from build123d import *

# Parameters (mm, degrees)
SKETCH3_W                                            = 50
SKETCH3_H                                            = 86
SKETCH3_R                                            = 14
BOSS_EXTRUDE1_DEPTH                                  = 21
M3_TAPPED_HOLE1_D                                    = 2.5
M3_TAPPED_HOLE1_DEPTH                                = 10
M3_TAPPED_HOLE1_TIP                                  = 0.751075774
BOSS_EXTRUDE3_START                                  = -2
SKETCH4_R                                            = 14
SKETCH4_R_2                                          = 12
BOSS_EXTRUDE3_DEPTH                                  = 2
F_4_0_4_DIAMETER_HOLE2_D                             = 4
SKETCH22_W                                           = 50
SKETCH22_H                                           = 15
BOSS_EXTRUDE5_DEPTH                                  = 20
SKETCH23_R                                           = 3.25
CUT_EXTRUDE3_DEPTH                                   = 92.989129793
F_4_0_4_DIAMETER_HOLE1_D                             = 4
F_4_0_4_DIAMETER_HOLE1_DEPTH                         = 15
F_4_0_4_DIAMETER_HOLE1_TIP                           = 1.201721238
HOLE_SIZE_PER_SOCKET_HEAD_CAP_SCREW_TYPE_D           = 4.5
HOLE_SIZE_PER_SOCKET_HEAD_CAP_SCREW_TYPE_CBORE_D     = 8
HOLE_SIZE_PER_SOCKET_HEAD_CAP_SCREW_TYPE_CBORE_DEPTH = 4.6
CHAMFER1_SIZE                                        = 3
CHAMFER2_SIZE                                        = 1


with BuildPart() as part:
    # Sketch3 → Boss-Extrude1 (new body)
    with BuildSketch(Plane.XY):
        with Locations((0, 43)):
            Rectangle(SKETCH3_W, SKETCH3_H)
        with Locations(Location((0, 60, 0), (0, 0, 180))):
            Circle(SKETCH3_R, mode=Mode.SUBTRACT)
    extrude(amount=BOSS_EXTRUDE1_DEPTH)

    # M3 Tapped Hole1
    with Locations(Plane(origin=(6.398868237, 17.925711715, 0), x_dir=(1, 0, 0), z_dir=(0, 0, -1))):
        with Locations((11.601131763, -42.074288285), (-24.398868237, -42.074288285)):
            Hole(M3_TAPPED_HOLE1_D / 2, depth=M3_TAPPED_HOLE1_DEPTH)
            with Locations((0, 0, -(M3_TAPPED_HOLE1_DEPTH + M3_TAPPED_HOLE1_TIP / 2))):  # 118° drill point
                Cone(0, M3_TAPPED_HOLE1_D / 2, M3_TAPPED_HOLE1_TIP, mode=Mode.SUBTRACT)

    # Sketch4 → Boss-Extrude3 (add)
    with BuildSketch(Plane.XY.offset(21).offset(BOSS_EXTRUDE3_START)):
        with Locations(Location((0, 60, 0), (0, 0, 180))):
            Circle(SKETCH4_R)
        with Locations((0, 60)):
            Circle(SKETCH4_R_2, mode=Mode.SUBTRACT)
    extrude(amount=BOSS_EXTRUDE3_DEPTH)

    # Ø4.0 (4) Diameter Hole2 (through all)
    with Locations(Plane.XY.offset(21)):
        with Locations((0, 81), (0, 39)):
            Hole(F_4_0_4_DIAMETER_HOLE2_D / 2)

    # Sketch22 → Boss-Extrude5 (add)
    with BuildSketch(Plane(origin=(0, 0, 0), x_dir=(-1, 0, 0), z_dir=(0, 0, -1))):
        with Locations((0, 7.5)):
            Rectangle(SKETCH22_W, SKETCH22_H)
    extrude(amount=BOSS_EXTRUDE5_DEPTH)

    # Sketch23 → Cut-Extrude3 (cut, through all)
    with BuildSketch(Plane.XZ):
        with Locations((12.5, -12)):
            Circle(SKETCH23_R)
        with Locations((-12.5, -12)):
            Circle(SKETCH23_R)
    extrude(amount=-CUT_EXTRUDE3_DEPTH, mode=Mode.SUBTRACT)

    # Ø4.0 (4) Diameter Hole1
    with Locations(Plane.XZ):
        with Locations((0, -15), (0, -5)):
            Hole(F_4_0_4_DIAMETER_HOLE1_D / 2, depth=F_4_0_4_DIAMETER_HOLE1_DEPTH)
            with Locations((0, 0, -(F_4_0_4_DIAMETER_HOLE1_DEPTH + F_4_0_4_DIAMETER_HOLE1_TIP / 2))):  # 118° drill point
                Cone(0, F_4_0_4_DIAMETER_HOLE1_D / 2, F_4_0_4_DIAMETER_HOLE1_TIP, mode=Mode.SUBTRACT)

    # Hole size per socket head cap screw type 1 (through all)
    with Locations(Plane(origin=(0, 0, 0), x_dir=(-1, 0, 0), z_dir=(0, 0, -1))):
        with Locations((-20, 80), (-20, 40), (20, 40), (20, 80)):
            CounterBoreHole(HOLE_SIZE_PER_SOCKET_HEAD_CAP_SCREW_TYPE_D / 2, HOLE_SIZE_PER_SOCKET_HEAD_CAP_SCREW_TYPE_CBORE_D / 2, HOLE_SIZE_PER_SOCKET_HEAD_CAP_SCREW_TYPE_CBORE_DEPTH)

    # Chamfer1
    chamfer1_edges = [part.edges().sort_by_distance(p)[0] for p in [
        (-25, 86, 10.5),
        (25, 86, 10.5),
    ]]
    chamfer(chamfer1_edges, length=CHAMFER1_SIZE)

    # Chamfer2
    chamfer2_edges = [part.edges().sort_by_distance(p)[0] for p in [
        (0, 0, 21),
        (25, 7.5, -20),
        (-25, 7.5, -20),
    ]]
    chamfer(chamfer2_edges, length=CHAMFER2_SIZE)


solid = part.part
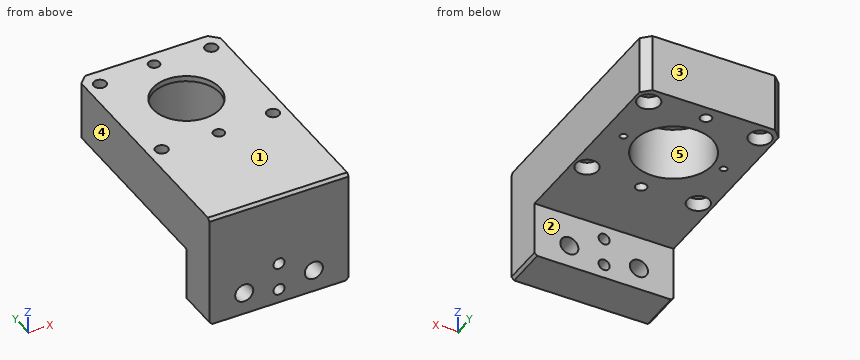
CAD build for the part. Positions are in the model's coordinates, mm. Face numbers are marked on the shaded views. A direction names the side the tool comes from. Coordinates: 2 decimals unless noted, no trailing zeros. Order: outer loops, then holes, each group sorted by start corner. A loop starts at its lowest first (then second) coordinate and runs counter-clockwise, first axis right, second up.
Item 1: Band-saw the part on C-C on z = -5. List the corners of the cut face in (x, y), plus the area to 3 significant figures.
Check sheet entries:
outline: (-25, 0) - (-2, 0) - (-2, 15) - (-25, 15) - close; (2, 0) - (25, 0) - (25, 15) - (2, 15) - close
area: 690 mm2
Item 2: Band-saw the part on A-A on y = 7. List the corners of the cut face in (x, z).
Check sheet entries:
outline: (-25, -19) - (-24, -20) - (24, -20) - (25, -19) - (25, 21) - (-25, 21) - close; hole circle Ø6.5 at (-12.5, -12); hole circle Ø4 at (0, -15); hole circle Ø4 at (0, -5); hole circle Ø6.5 at (12.5, -12)
Item 3: Pin check, flat tips, straight feed: pin 1 Ø4 at (x, y) = (20, 80) entering from +Z; pin 2 Ø4 at (x, z) = (-10.5, -4.5) entering from +Y; pin 3 Ø1 at (x, y) = (9, 26) entering from -Z; pin 4 Ø2.5 at (x, y) = (-18.5, 41.5) entering from -Z. Stop position of each tip, or through.
Check sheet entries:
pin 1: passes through
pin 2: stops at y = 15
pin 3: stops at z = 0
pin 4: stops at z = 4.6
Item 4: Two-plate mould, pull along X, no slides. Class the marked faces 3, 4 and 5: +X half, -X half, draft (parallel to the pull), parting line (faces both ways), or undercut.
Check sheet entries:
face 3: draft
face 4: -X half
face 5: undercut
Item 5: Band-saw the part on D-D on x = 8. List the corners of the cut face in (y, z).
Check sheet entries:
outline: (0, -20) - (15, -20) - (15, 0) - (48.51, 0) - (48.51, 19) - (51.06, 19) - (51.06, 21) - (1, 21) - (0, 20) - close; (68.94, 19) - (71.49, 19) - (71.49, 0) - (86, 0) - (86, 21) - (68.94, 21) - close
Item 6: Band-saw the part on B-B on x = 0. Give the number of separate pieces and of enclosed holes in the cut face, plus the area to 3 significant figures.
Check sheet entries:
separate pieces: 6
enclosed holes: 0
area: 1,240 mm2
Item 7: Drill centre lines: L1, parallel to Y at x = 0, z = 10.5; L2, parallel to Y at x = 20, z = 2.5; L3, parallel to Z at x = 12.5, y = 8.25. Where is each one in solid material? Low to high.
Check sheet entries:
L1: y = 0 to 37, 41 to 46, 74 to 79, 83 to 86
L2: y = 0 to 36, 44 to 76, 84 to 86
L3: z = -20 to -15.25, -8.75 to 21
Item 8: 3-axis set-ups, long thin cutter, end or side, ignore diameter. For the marked faces 1 and 2: which of +Z, -Z, +X, -X, +Y, -Y reach the whole face in a straight line?
Check sheet entries:
face 1: +Z, +X, -X, +Y, -Y
face 2: -Z, +X, -X, +Y
